The model under review builds one solid part; all positions refer to its coordinate system, in mm. Face numbers are marked on the shaded views. A direction names the side the tool comes from. Round coordinates to 2 decimals unless told otherwise and drop trailing zeros. Order: outer loops, then holes, each group sorted by start corner. A loop starts at its lowest first (then second) coordinate and runs counter-clockwise, first axis right, second up. Notation, with made-up numbers: (21, 76.25) -> (48, 76.25) arc R9 ccw to (48, 80.25) -> close; hole circle Ø8 at (89.25, -22). An arc over 180 degrees is marked (long way). Use a Markdown table: item, result. Add a question column.
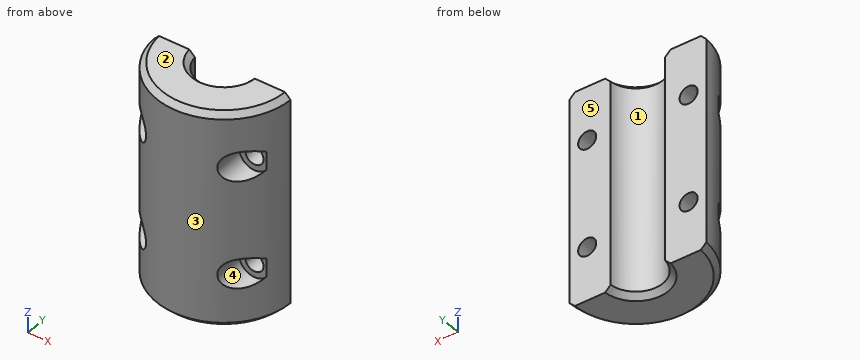
```python
from build123d import *

# Parameters (mm, degrees)
EXTRUDE_1_DEPTH           = 80
SKETCH_2_R                = 5.5
CUT_EXTRUDE_1_DEPTH       = 100
HOLE_WIZARD_1_D           = 6.6
HOLE_WIZARD_1_CBORE_D     = 11
HOLE_WIZARD_1_CBORE_DEPTH = 6.8
CHAMFER_1_SIZE            = 2


with BuildPart() as part:
    # 草图1 → 凸台-拉伸1 (new body)
    with BuildSketch(Plane.XY):
        with BuildLine():
            Line((-24.979991994, -1), (-9.949874371, -1))
            ThreePointArc((-9.949874371, -1), (0, -10), (9.949874371, -1))
            Line((9.949874371, -1), (24.979991994, -1))
            ThreePointArc((24.979991994, -1), (0, -25), (-24.979991994, -1))
        make_face()
    extrude(amount=EXTRUDE_1_DEPTH)

    # 草图2 → 切除-拉伸1 (cut)
    with BuildSketch(Plane(origin=(0, -17, 0), x_dir=(1, 0, 0), z_dir=(0, 1, 0))):
        with Locations((-18.5, -20)):
            Circle(SKETCH_2_R)
        with Locations((18.5, -20)):
            Circle(SKETCH_2_R)
        with Locations((18.5, -60)):
            Circle(SKETCH_2_R)
        with Locations((-18.5, -60)):
            Circle(SKETCH_2_R)
    extrude(amount=-CUT_EXTRUDE_1_DEPTH, mode=Mode.SUBTRACT)

    # 打孔尺寸(%根据)内六角圆柱头螺钉的类型1 (through all)
    with Locations(Plane(origin=(0, -17, 0), x_dir=(-1, 0, 0), z_dir=(0, -1, 0))):
        with Locations((-18.5, -20), (18.5, -20), (18.5, -60), (-18.5, -60)):
            CounterBoreHole(HOLE_WIZARD_1_D / 2, HOLE_WIZARD_1_CBORE_D / 2, HOLE_WIZARD_1_CBORE_DEPTH)

    # 倒角1
    chamfer_1_edges = [part.edges().sort_by_distance(p)[0] for p in [
        (0, -25, 80),
        (0, -10, 80),
        (0, -25, 0),
        (0, -10, 0),
    ]]
    chamfer(chamfer_1_edges, length=CHAMFER_1_SIZE)


solid = part.part
```
Q1. Add section B-B, the plane x = 0. Give the boundary of the cut face in (y, z).
Q2. Add section D-D, the plane z = 30. Give the boundary of the cut face in (x, y), then the cut area to 3 significant figures.
Q3. To check wall thickness, follow line 1 along Z through (x, y) = (18.5, -7.25); line 2 along X through (y, z) = (-7.5, 20); line 3 along X through (y, z) = (-4.25, 60). State the ranges of each line that lie inside material, in increasing order.
Q4. Draft analysis for pull direction X (two halves, no side actions). For the marked faces 1, 2 and 3, state which applies: released by +X, released by -X, zero draft, split by the parting line, or undercut.
Q5. Add section C-C, the plane y = -3.5. Give the number of separate pieces and of enclosed holes in the cut face, then the cut area to 3 significant figures.
Q6. For pin 1 (2 mm diameter, centred on x = 5.5, z = 45.5, fed in from +Y); pin 2 (10 mm diameter, centred on y = -10.5, z = 48, fed in from -X); pin 3 (5 mm diameter, centred on x = -18, z = 21.5, fed in from -Y), all flat-tipped, find the tip position at first contact; note any pin that passes through.
Q7. For the marked faces 4 and 5, list the 3-axis set-ups (+Z, -Z, +X, -X, +Y, -Y) from which the entire face can be reached by the end or side of a thin tool; tool diameter is ignored.
Q8. Add section A-A, the plane z = 20. Give the boundary of the cut face in (x, y), then the cut area to 3 significant figures.
Return value:
| question | item | result |
|---|---|---|
| 1 | outline | (-25, 2) -> (-23, 0) -> (-12, 0) -> (-10, 2) -> (-10, 78) -> (-12, 80) -> (-23, 80) -> (-25, 78) -> close |
| 2 | outline | (-24.98, -1) arc R25 ccw to (24.98, -1) -> (9.95, -1) arc R10 cw to (-9.95, -1) -> close |
| 2 | area | 795 mm² |
| 3 | line 1 | 0 to 16.7, 23.3 to 56.7, 63.3 to 80 |
| 3 | line 2 | -23.85 to -21.8, -15.2 to -6.61, 6.61 to 15.2, 21.8 to 23.85 |
| 3 | line 3 | -24.64 to -21.8, -15.2 to -9.05, 9.05 to 15.2, 21.8 to 24.64 |
| 4 | face 1 | undercut |
| 4 | face 2 | zero draft |
| 4 | face 3 | split by the parting line |
| 5 | separate pieces | 2 |
| 5 | enclosed holes | 4 |
| 5 | area | 2,310 mm² |
| 6 | pin 1 | y = -7.6 |
| 6 | pin 2 | x = -24.39 |
| 6 | pin 3 | y = -10.2 |
| 7 | face 4 | -Y |
| 7 | face 5 | +Z, -Z, +X, -X, +Y |
| 8 | outline | (-24.98, -1) arc R25 ccw to (-22.82, -10.2) -> (-21.8, -10.2) -> (-21.8, -1) -> close; (-15.2, -10.2) -> (-13, -10.2) -> (-13, -21.35) arc R25 ccw to (13, -21.35) -> (13, -10.2) -> (15.2, -10.2) -> (15.2, -1) -> (9.95, -1) arc R10 cw to (-9.95, -1) -> (-15.2, -1) -> close; (21.8, -10.2) -> (22.82, -10.2) arc R25 ccw to (24.98, -1) -> (21.8, -1) -> close |
| 8 | area | 541 mm² |
